Design review of the part built by this model. Coordinates are the model's own, in mm. Face numbers are marked on the shaded views. A direction names the side the tool comes from. Round coordinates to 2 decimals unless told otherwise and drop trailing zeros. Loops run counter-clockwise (first coordinate to the right, second up) from the corner with the lowest first, then second, coordinate; pieces in that order, holes last. Notation, with made-up numbers: (89, 55) -> (117, 55) arc R19 ccw to (117, 76) -> close; hole circle Ø2 at (-2.5, 8.25). An arc over 180 degrees is marked (long way). Answer as CSV lines item,"result". Start each with the question number.
(1) For P1, Ø25, axis at x = 22.5, y = 2, coming from the +Z side; P2, Ø6, axis at x = -33.5, z = 28.5, coming from the +Y side; P3, Ø3, axis at x = -60, z = 92.5, coming from the +Y side, all flat-tipped, find the tip position at first contact; note any pin that passes through.
(2) To check wall thickness, follow line 1 (Y direction, x = 37, z = 6); line 2 (Y direction, x = 0, z = 7.5); line 3 (Z direction, x = 15.5, y = -4). State the ranges of each line that lie inside material, in increasing order. Write a range as from..to.
(3) Take a section at A-A, the plane x = -37.5. Write out the cut boundary in (y, z), and give its area (3 significant figures).
(4) Take a section at C-C, the plane y = -20. Write out the cut boundary in (x, z).
(5) Draft analysis for pull direction X (two halves, no side actions). For the marked faces 1, 2, 3 and 4, state which applies: +X half, -X half, draft (parallel to the pull), parting line (faces both ways), or undercut.
(6) Take a section at B-B, the plane x = 60. Write out the cut boundary in (y, z).
(7) Machinability: for the marked faces 5 and 6, which of the approach directions +Z, -Z, +X, -X, +Y, -Y give a long, thin tool a straight path to every point of the face, cutting with its end or side? Answer none if there is none.
(8) Take a section at D-D, the plane z = 24. Write out the cut boundary in (x, y).
from build123d import *

# Parameters (mm, degrees)
SKETCH1_W                  = 200
SKETCH1_H                  = 50
SKETCH1_R                  = 11.5
BOSS_EXTRUDE1_DEPTH        = 12.5
SKETCH2_W                  = 200
SKETCH2_H                  = 100
BOSS_EXTRUDE2_DEPTH        = 6
M8X1_25_TAPPED_HOLE1_D     = 6.8
M8X1_25_TAPPED_HOLE1_DEPTH = 19.75
M8X1_25_TAPPED_HOLE1_TIP   = 2.042926105
SKETCH6_R                  = 5
BOSS_EXTRUDE3_DEPTH        = 40
SKETCH7_R                  = 7.408343544
SKETCH7_R_2                = 4
SKETCH7_R_3                = 9.473582921
CUT_EXTRUDE1_DEPTH         = 1
SKETCH8_R                  = 11.635219883
SKETCH8_R_2                = 4
SKETCH8_R_3                = 12.853619102
CUT_EXTRUDE2_DEPTH         = 1
CUT_EXTRUDE3_REACH         = 154.105
SKETCH9_W                  = 25
SKETCH9_H                  = 100


with BuildPart() as part:
    # Sketch1 → Boss-Extrude1 (new body)
    with BuildSketch(Plane.XY):
        Rectangle(SKETCH1_W, SKETCH1_H)
        Circle(SKETCH1_R, mode=Mode.SUBTRACT)
    extrude(amount=BOSS_EXTRUDE1_DEPTH)

    # Sketch2 → Boss-Extrude2 (add)
    with BuildSketch(Plane.XZ.offset(25)):
        with Locations((0, 50)):
            Rectangle(SKETCH2_W, SKETCH2_H)
    extrude(amount=BOSS_EXTRUDE2_DEPTH)

    # M8x1.25 Tapped Hole1
    with Locations(Plane(origin=(37.5, 0, 0), x_dir=(-1, 0, 0), z_dir=(0, 0, -1))):
        with Locations((0, 0), (75, 0)):
            Hole(M8X1_25_TAPPED_HOLE1_D / 2, depth=M8X1_25_TAPPED_HOLE1_DEPTH)
            with Locations((0, 0, -(M8X1_25_TAPPED_HOLE1_DEPTH + M8X1_25_TAPPED_HOLE1_TIP / 2))):  # 118° drill point
                Cone(0, M8X1_25_TAPPED_HOLE1_D / 2, M8X1_25_TAPPED_HOLE1_TIP, mode=Mode.SUBTRACT)

    # Sketch6 → Boss-Extrude3 (add)
    with BuildSketch(Plane(origin=(0, -25, 0), x_dir=(1, 0, 0), z_dir=(0, 1, 0))):
        with Locations(Location((60, -92.5, 0), (0, 0, 270))):
            Circle(SKETCH6_R)
        with Locations(Location((-60, -92.5, 0), (0, 0, 270))):
            Circle(SKETCH6_R)
    extrude(amount=BOSS_EXTRUDE3_DEPTH)

    # Sketch7 → Cut-Extrude1 (cut)
    # profile 1 of 2: a face of its own
    with BuildSketch(Plane(origin=(0, 10.5, 0), x_dir=(1, 0, 0), z_dir=(0, 1, 0))):
        with Locations((60, -92.5)):
            Circle(SKETCH7_R)
        with Locations(Location((60, -92.5, 0), (0, 0, 270))):
            Circle(SKETCH7_R_2, mode=Mode.SUBTRACT)
    # profile 2 of 2: a face of its own
    with BuildSketch(Plane(origin=(0, 10.5, 0), x_dir=(1, 0, 0), z_dir=(0, 1, 0))):
        with Locations((-60, -92.5)):
            Circle(SKETCH7_R_3)
        with Locations(Location((-60, -92.5, 0), (0, 0, 270))):
            Circle(SKETCH7_R_2, mode=Mode.SUBTRACT)
    extrude(amount=-CUT_EXTRUDE1_DEPTH, mode=Mode.SUBTRACT)

    # Sketch8 → Cut-Extrude2 (cut)
    # profile 1 of 2: a face of its own
    with BuildSketch(Plane(origin=(0, -10, 0), x_dir=(1, 0, 0), z_dir=(0, 1, 0))):
        with Locations((60, -92.5)):
            Circle(SKETCH8_R)
        with Locations(Location((60, -92.5, 0), (0, 0, 270))):
            Circle(SKETCH8_R_2, mode=Mode.SUBTRACT)
    # profile 2 of 2: a face of its own
    with BuildSketch(Plane(origin=(0, -10, 0), x_dir=(1, 0, 0), z_dir=(0, 1, 0))):
        with Locations((-60, -92.5)):
            Circle(SKETCH8_R_3)
        with Locations(Location((-60, -92.5, 0), (0, 0, 270))):
            Circle(SKETCH8_R_2, mode=Mode.SUBTRACT)
    extrude(amount=-CUT_EXTRUDE2_DEPTH, mode=Mode.SUBTRACT)

    # Sketch9 → Cut-Extrude3 (cut, up to next)
    with BuildSketch(Plane.XZ.offset(31), mode=Mode.PRIVATE) as cut_extrude3_sk1:
        with Locations((87.5, 50)):
            Rectangle(SKETCH9_W, SKETCH9_H)
    cut_extrude3_tool1 = extrude(cut_extrude3_sk1.sketch, amount=-CUT_EXTRUDE3_REACH, mode=Mode.PRIVATE) & part.part
    # Sketch9 → Cut-Extrude3 (cut, up to next)
    with BuildSketch(Plane.XZ.offset(31), mode=Mode.PRIVATE) as cut_extrude3_sk2:
        with Locations((-87.5, 50)):
            Rectangle(SKETCH9_W, SKETCH9_H)
    cut_extrude3_tool2 = extrude(cut_extrude3_sk2.sketch, amount=-CUT_EXTRUDE3_REACH, mode=Mode.PRIVATE) & part.part
    add(cut_extrude3_tool1.solids().sort_by_distance((87.5, -31, 50))[0], mode=Mode.SUBTRACT)
    add(cut_extrude3_tool2.solids().sort_by_distance((-87.5, -31, 50))[0], mode=Mode.SUBTRACT)


solid = part.part
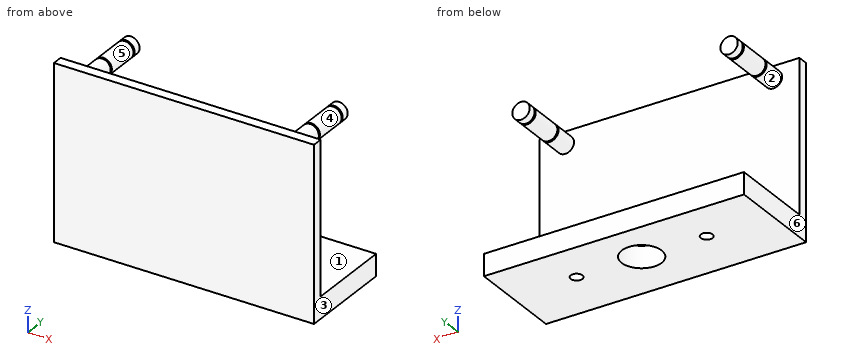
The answers:
1,P1,"z = 12.5"
1,P2,"y = -25"
1,P3,"y = 15"
2,line 1,"-31..-3.36, 3.36..25"
2,line 2,"-31..-11.5, 11.5..25"
2,line 3,"0..12.5"
3,outline,"(-31, 0) -> (-3.4, 0) -> (-3.4, 12.5) -> (-25, 12.5) -> (-25, 100) -> (-31, 100) -> close; (3.4, 0) -> (25, 0) -> (25, 12.5) -> (3.4, 12.5) -> close"
3,area,"1,140 mm²"
4,outline,"(-75, 0) -> (75, 0) -> (75, 12.5) -> (-75, 12.5) -> close; circle Ø10 at (-60, 92.5); circle Ø10 at (60, 92.5)"
5,face 1,"draft"
5,face 2,"undercut"
5,face 3,"+X half"
5,face 4,"undercut"
6,outline,"(-31, 0) -> (25, 0) -> (25, 12.5) -> (-25, 12.5) -> (-25, 87.5) -> (-11, 87.5) -> (-11, 88.5) -> (-10, 88.5) -> (-10, 87.5) -> (9.5, 87.5) -> (9.5, 88.5) -> (10.5, 88.5) -> (10.5, 87.5) -> (15, 87.5) -> (15, 97.5) -> (10.5, 97.5) -> (10.5, 96.5) -> (9.5, 96.5) -> (9.5, 97.5) -> (-10, 97.5) -> (-10, 96.5) -> (-11, 96.5) -> (-11, 97.5) -> (-25, 97.5) -> (-25, 100) -> (-31, 100) -> close"
7,face 5,"+Y"
7,face 6,"+Z, -Z, -X, +Y, -Y"
8,outline,"(-75, -31) -> (75, -31) -> (75, -25) -> (-75, -25) -> close"
